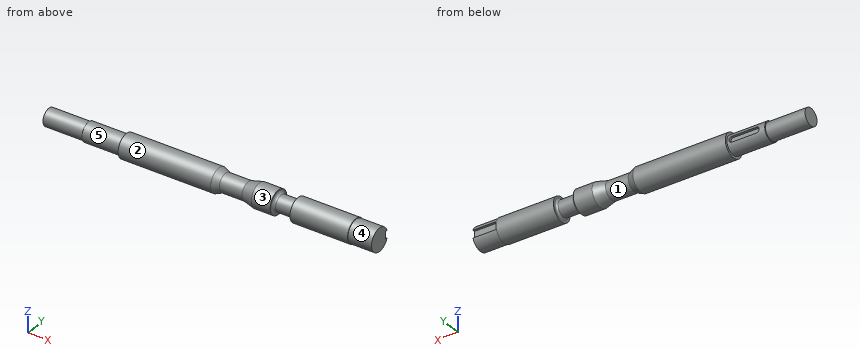
```python
from build123d import *

# Parameters (mm, degrees)
SHOULDER_FILLET_R2_R    = 2
SHOULDER_FILLET_R3_R    = 3
KEYWAY_A_SKETCH_W       = 8
KEYWAY_A_SKETCH_H       = 6
KEYWAY_A_CUT_DEPTH      = 25
KEYWAY_START            = 10
KEYWAY_B_CUT_26X3_DEPTH = 3


with BuildPart() as part:
    # Shaft Profile Sketch → Shaft Body Revolve (revolve)
    with BuildSketch(Plane.XY, mode=Mode.PRIVATE) as shaft_body_revolve_sk:
        Polygon((0, 0), (350, 0), (350, 12), (325, 12), (325, 12.5), (264, 12.5), (264, 8.5), (243, 8.5), (243, 12.5), (223, 12.5), (211, 9.5), (187, 9.5), (180, 12.5), (82, 12.5), (82, 10), (42, 10), (42, 9), (0, 9), align=None)
    revolve(shaft_body_revolve_sk.sketch.rotate(Axis((0, 0, 0), (1, 0, 0)), 90), axis=Axis((0, 0, 0), (1, 0, 0)))

    # Shoulder Fillet R2
    shoulder_fillet_r2_edges = [part.edges().sort_by_distance(p)[0] for p in [
        (264, 0, -8.5),
    ]]
    fillet(shoulder_fillet_r2_edges, radius=SHOULDER_FILLET_R2_R)

    # Shoulder Fillet R3
    shoulder_fillet_r3_edges = [part.edges().sort_by_distance(p)[0] for p in [
        (243, 0, -8.5),
    ]]
    fillet(shoulder_fillet_r3_edges, radius=SHOULDER_FILLET_R3_R)

    # Keyway A Sketch → Keyway A Cut (cut)
    with BuildSketch(Plane(origin=(350, 0, 0), x_dir=(0, 0, -1), z_dir=(1, 0, 0))):
        with Locations((0, 12)):
            Rectangle(KEYWAY_A_SKETCH_W, KEYWAY_A_SKETCH_H)
    extrude(amount=-KEYWAY_A_CUT_DEPTH, mode=Mode.SUBTRACT)

    # Keyway B Sketch 26x3 → Keyway B Cut 26x3 (cut)
    with BuildSketch(Plane(origin=(0, 0, 0), x_dir=(1, 0, 0), z_dir=(0, 1, 0)).offset(KEYWAY_START)):
        with BuildLine():
            Line((51, 3), (77, 3))
            ThreePointArc((77, 3), (80, 0), (77, -3))
            Line((77, -3), (51, -3))
            ThreePointArc((51, -3), (48, 0), (51, 3))
        make_face()
    extrude(amount=-KEYWAY_B_CUT_26X3_DEPTH, mode=Mode.SUBTRACT)


solid = part.part
```
For this review, take the finished solid that the model builds, in its own axes (mm). Face numbers are marked on the shaded views. A direction names the side the tool comes from. Round coordinates to 2 decimals unless told otherwise and drop trailing zeros. Write each loop counter-clockwise with the first axis right and the second up, starting at its lowest first coordinate (ties: lowest second). Pieces come first, ordered by that corner, then holes.
1) Take a section at A-A on x = 69.5. Give the boundary of the cut face in (y, z).
Answer below:
outline: (7, -3) - (7, 3) - (9.54, 3) arc R10 ccw (long way) to (9.54, -3) - close
2) Mouldability with a two-part tool opening along X and no side actions: class the marked faces 1 and 2 as +X half, -X half, draft (parallel to the pull), parting line (faces both ways), or undercut.
Answer below:
face 1: undercut
face 2: draft
3) Insertion check: pin 1 Ø3 at (x, z) = (74, 6) entering from +Y; pin 2 Ø9 at (x, z) = (335.5, 0) entering from +Y; pin 3 Ø3 at (x, z) = (36.5, 9.5) entering from +Y. Each pin has a flat end and moves straight along its axis. Give the tip position at first contact, or say it passes through.
Answer below:
pin 1: stops at y = 8.93
pin 2: stops at y = 11.31
pin 3: stops at y = 4.12
4) For line 1 along Y through (x, z) = (219, -0.5); line 2 along Y through (x, z) = (239.5, 0.75); line 3 along Z through (x, y) = (301, 3.25), list the stretches that pass through material, from the lowest coordinate up.
Answer below:
line 1: y = -11.49 to 11.49
line 2: y = -12.48 to 12.48
line 3: z = -12.07 to 12.07
5) Machinability: for the marked faces 3, 4 and 5, which of the approach directions +Z, -Z, +X, -X, +Y, -Y give a long, thin tool a straight path to every point of the face, cutting with its end or side? Answer none if there is none.
Answer below:
face 3: +X, -X
face 4: +X
face 5: -X
